Check sheet for the drawn part. Datum: minimum x, y, z corner. Units: mm. A direction names the side the tool comes from. Round coordinates to 2 decimals unless told otherwise and drop trailing zeros. Write each loop counter-clockwise with the first axis right and the second up, starting at its lowest first coordinate (ties: lowest second). Pieces come first, ordered by that corner, then holes. Notation, with made-up numbers: M -38,51.5 L 21,51.5 A25 cw 21,78.5 Z; hole C 16,-21 d4. An arc over 180 degrees is marked long. Use a Markdown table: item, result.
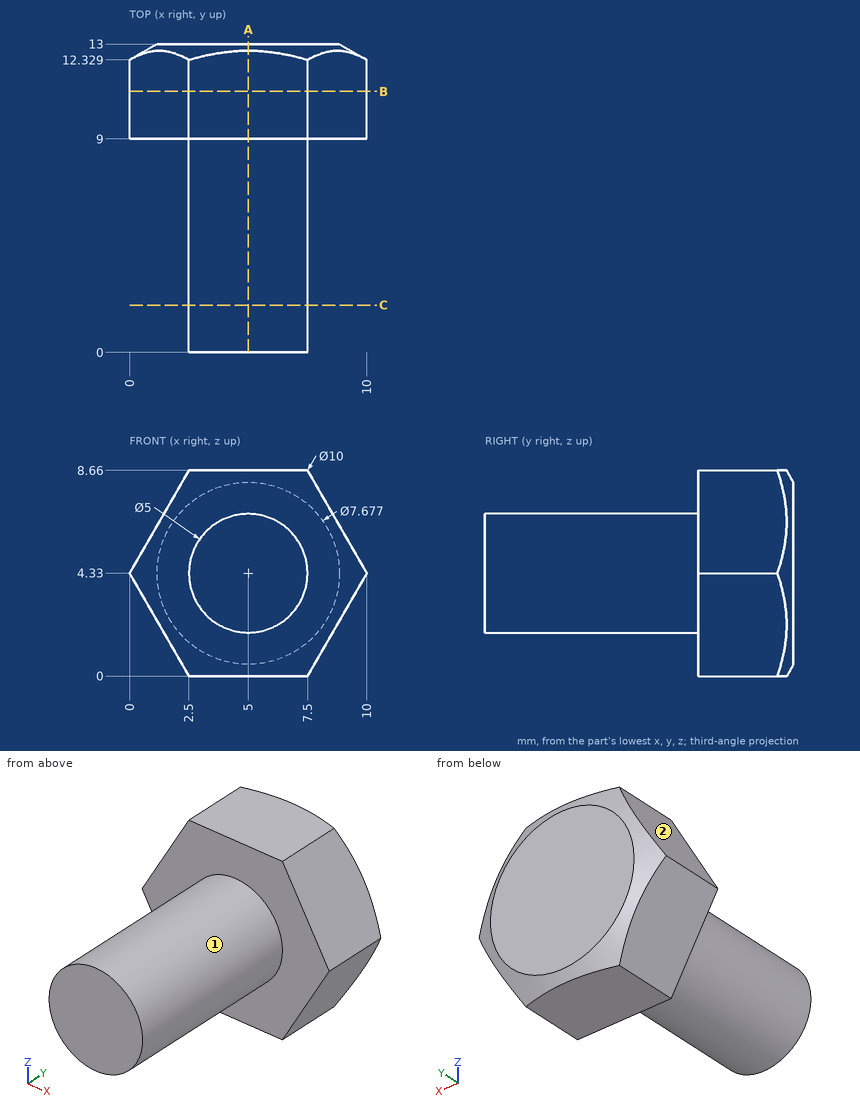
Item 1: Cross-section at B-B, the plane y = 11. Record the cut outline in (x, z).
Outcome:
| item | result |
|---|---|
| outline | M 0,4.33 L 2.5,0 L 7.5,0 L 10,4.33 L 7.5,8.66 L 2.5,8.66 Z |
Item 2: Material ranges on line 1 along X through (y, z) = (10.75, 7.5); line 2 along X through (y, z) = (4.75, 5); line 3 along Z through (x, y) = (6.75, 8) (1 decimal), recorded low to high. Write a range as from..to.
Outcome:
| item | result |
|---|---|
| line 1 | x = 1.83..8.17 |
| line 2 | x = 2.59..7.41 |
| line 3 | z = 2.5..6.1 |
Item 3: Cross-section at A-A, the plane x = 5. Record the cut outline in (y, z), and give its area (3 significant figures).
Outcome:
| item | result |
|---|---|
| outline | M 0,1.83 L 9,1.83 L 9,0 L 12.72,0 L 13,0.49 L 13,8.17 L 12.72,8.66 L 9,8.66 L 9,6.83 L 0,6.83 Z |
| area | 79.5 mm2 |
Item 4: Go/stop test with flat-tipped pins: pin 1 (2.5 mm diameter, centred on x = 5.5, z = 3.5, fed in from -Y); pin 2 (1 mm diameter, centred on y = 4.5, z = 5, fed in from -X); pin 3 (6 mm diameter, centred on x = 1.5, y = 3, fed in from -Z). Record where each tip stops, or that it passes through.
Outcome:
| item | result |
|---|---|
| pin 1 | stops at y = 0 |
| pin 2 | stops at x = 2.51 |
| pin 3 | stops at z = 1.88 |
Item 5: Access from +Z, -Z, +X, -X, +Y, -Y to the whole of each face (thin tool, end or side, straight path). Record for the marked faces 1 and 2.
Outcome:
| item | result |
|---|---|
| face 1 | -Y |
| face 2 | +Z, -X, +Y, -Y |
Item 6: Cross-section at C-C, the plane y = 2. Record the cut outline in (x, z), and give its area (3 significant figures).
Outcome:
| item | result |
|---|---|
| outline | C 5,4.33 d5 |
| area | 19.6 mm2 |
